Can you work these out from the model? Positions are in its coordinate system, mm. Coordinates: 2 decimals unless noted, no trailing zeros. Loops run counter-clockwise (first coordinate to the right, second up) from the corner with the lowest first, then second, coordinate; pieces in that order, holes last. Notation, with made-up numbers: M 57,29.5 L 108,29.5 A19 cw 108,49.5 Z; hole C 2.25,-9 d1. An arc over 180 degrees is marked long. Answer as a JSON object with one key per item and string values. Group by question number.
Item 1: We'd pull the mould along Y, two halves only. Please class faces 1 (the flat face through (-11, -82, 0)), 2 (the cylindrical face through (-135.59, 89.46, 1.52)): +Y half, -Y half, draft (parallel to the pull), parting line (faces both ways), or undercut.
Item 2: Suppose I cut it at C-C (z = 1.05). Write out the boundary of the cut face in (x, y), then the cut area to 3 significant figures.
Item 3: I'm going to push a flat-ended pin straight in: pin 1 Ø8 at (x, y) = (-135, -85) entering from +Z. Where does the tip first touch, or does it pass through?
Item 4: Suppose I cut it at D-D (x = 2.5). Write out the boundary of the cut face in (y, z).
Item 5: If I drill on line 1 (Y direction, x = -135, z = 0.7); line 2 (X direction, y = 51.5, z = 2.7); line 3 (Y direction, x = 62, z = 2.1), over which ranges is the centre line in solid material (lowest first)?
Item 6: Suppose I cut it at B-B (y = -85). Write out the boundary of the cut face in (x, z).
Item 7: Suppose I cut it at A-A (x = 135). Write out the boundary of the cut face in (y, z), then the cut area to 3 significant figures.
```python
from build123d import *

# Parameters (mm, degrees)
SKETCH1_W            = 290
SKETCH1_H            = 185
SKETCH1_W_2          = 260
SKETCH1_H_2          = 157
BOSS_EXTRUDE1_DEPTH  = 3
SKETCH2_R            = 4.5
CUT_EXTRUDE1_DEPTH   = 3
LPATTERN1_COUNT      = 2
LPATTERN1_PITCH      = 270
LPATTERN1_COUNT_DIR2 = 2
LPATTERN1_PITCH_DIR2 = 170


with BuildPart() as part:
    # Sketch1 → Boss-Extrude1 (new body)
    with BuildSketch(Plane.XY):
        Rectangle(SKETCH1_W, SKETCH1_H)
        Rectangle(SKETCH1_W_2, SKETCH1_H_2, mode=Mode.SUBTRACT)
    extrude(amount=BOSS_EXTRUDE1_DEPTH)

    # Sketch2 → Cut-Extrude1 (cut)
    with BuildSketch(Plane.XY.offset(3)):
        with Locations((-135, 85)):
            Circle(SKETCH2_R)
    cut_extrude1 = extrude(amount=-CUT_EXTRUDE1_DEPTH, mode=Mode.SUBTRACT)

    # LPattern1: Cut-Extrude1 2 × 2
    with Locations(*[(i * LPATTERN1_PITCH, -j * LPATTERN1_PITCH_DIR2, 0) for i in range(LPATTERN1_COUNT) for j in range(LPATTERN1_COUNT_DIR2) if (i, j) != (0, 0)]):
        add(cut_extrude1, mode=Mode.SUBTRACT)


solid = part.part
```
From the geometry:
{
 "1": {"face 1": "draft", "face 2": "undercut"},
 "2": {"outline": "M -145,-92.5 L 145,-92.5 L 145,92.5 L -145,92.5 Z; hole C -135,-85 d9; hole C -135,85 d9; hole M -130,-78.5 L 130,-78.5 L 130,78.5 L -130,78.5 Z; hole C 135,-85 d9; hole C 135,85 d9", "area": "12,600 mm2"},
 "3": {"pin 1": "through"},
 "4": {"outline": "M -92.5,0 L -78.5,0 L -78.5,3 L -92.5,3 Z; M 78.5,0 L 92.5,0 L 92.5,3 L 78.5,3 Z"},
 "5": {"line 1": "-92.5 to -89.5, -80.5 to 80.5, 89.5 to 92.5", "line 2": "-145 to -130, 130 to 145", "line 3": "-92.5 to -78.5, 78.5 to 92.5"},
 "6": {"outline": "M -145,0 L -139.5,0 L -139.5,3 L -145,3 Z; M -130.5,0 L 130.5,0 L 130.5,3 L -130.5,3 Z; M 139.5,0 L 145,0 L 145,3 L 139.5,3 Z"},
 "7": {"outline": "M -92.5,0 L -89.5,0 L -89.5,3 L -92.5,3 Z; M -80.5,0 L 80.5,0 L 80.5,3 L -80.5,3 Z; M 89.5,0 L 92.5,0 L 92.5,3 L 89.5,3 Z", "area": "501 mm2"}
}
